from build123d import *

# Parameters (mm, degrees)
BOSS_EXTRUDE1_DEPTH      = 10
BOSS_EXTRUDE1_DEPTH_BACK = 12
SKETCH1_W                = 70
SKETCH1_H                = 20
SKETCH1_R                = 2.187999439
SKETCH1_R_2              = 2.181063018
HOLE1_D                  = 6
HOLE1_CBORE_D            = 9.5
HOLE1_CBORE_DEPTH        = 8.5
CHAMFER1_SIZE            = 2


with BuildPart() as part:
    # Sketch1 → Boss-Extrude1 (new, two sides: drawn at the far end of the back side and taken through both)
    with BuildSketch(Plane.XY.offset(-BOSS_EXTRUDE1_DEPTH_BACK)):
        with Locations((2.309691162, 2.003205128)):
            Rectangle(SKETCH1_W, SKETCH1_H)
        with Locations((-24.690308838, 2.003205128)):
            Circle(SKETCH1_R, mode=Mode.SUBTRACT)
        with Locations((29.309691162, 2.003205128)):
            Circle(SKETCH1_R_2, mode=Mode.SUBTRACT)
    extrude(amount=BOSS_EXTRUDE1_DEPTH + BOSS_EXTRUDE1_DEPTH_BACK)

    # Hole1 (through all)
    with Locations(Plane.XY.offset(10)):
        with Locations((-24.690308838, 2.003205128), (29.309691162, 2.003205128)):
            CounterBoreHole(HOLE1_D / 2, HOLE1_CBORE_D / 2, HOLE1_CBORE_DEPTH)

    # Chamfer1
    chamfer1_edges = [part.edges().sort_by_distance(p)[0] for p in [
        (-32.690308838, 12.003205128, -1),
        (37.309691162, 12.003205128, -1),
        (37.309691162, -7.996794872, -1),
        (-32.690308838, -7.996794872, -1),
    ]]
    chamfer(chamfer1_edges, length=CHAMFER1_SIZE)


solid = part.part
Design review of the part built by this model. Coordinates are the model's own, in mm. A direction names the side the tool comes from. Coordinates: 2 decimals unless noted, no trailing zeros. Order: outer loops, then holes, each group sorted by start corner. A loop starts at its lowest first (then second) coordinate and runs counter-clockwise, first axis right, second up.
Item 1: Take a section at A-A, the plane y = 3.25. Write out the cut boundary in (x, z).
Item 2: For pin 1 Ø8 at (x, y) = (-24.69, 2) entering from +Z; pin 2 Ø5 at (x, y) = (-23, 0) entering from +Z, all flat-tipped, find the tip position at first contact; note any pin that passes through.
Item 3: The part is to be moulded in two halves that separate along Y. For faces 3 (the flat face through (-23.7, -1.1, 1.5)), 4 (the flat face through (-31.676, 11.017, -1.154)), 5 (the flat face through (-31.676, -7.011, -1.154)), say which applies: pulls with the +Y half, pulls with the -Y half, needs draft (parallel to the pull), parting line crosses it, or undercut.
Item 4: Take a section at C-C, the plane z = 3.5. Write out the cut boundary in (x, y).
Item 5: For line 1 (X direction, y = 1.25, z = 0); line 2 (X direction, y = 3, z = 9.25); line 3 (Z direction, x = 25, y = 3.25), list the stretches that pass through material, from the lowest coordinate up.
Item 6: For faces 1 (the cylindrical face through (26.54, 0.85, -5.34)), 2 (the cylindrical face through (25.54, -0.89, 5.81)), list the 3-axis set-ups (+Z, -Z, +X, -X, +Y, -Y) from which the entire face can be reached by the end or side of a thin tool; tool diameter is ignored.
Item 7: Take a section at B-B, the plane z = -3.75. Write out the cut boundary in (x, y).
The answers:
1. outline: (-32.69, -12) - (-27.42, -12) - (-27.42, 1.5) - (-29.27, 1.5) - (-29.27, 10) - (-32.69, 10) - close; (-21.96, -12) - (26.58, -12) - (26.58, 1.5) - (24.73, 1.5) - (24.73, 10) - (-20.11, 10) - (-20.11, 1.5) - (-21.96, 1.5) - close; (32.04, -12) - (37.31, -12) - (37.31, 10) - (33.89, 10) - (33.89, 1.5) - (32.04, 1.5) - close
2. pin 1: stops at z = 1.5
2. pin 2: stops at z = 10
3. face 3: undercut
3. face 4: pulls with the +Y half
3. face 5: pulls with the -Y half
4. outline: (-32.69, -6) - (-30.69, -8) - (35.31, -8) - (37.31, -6) - (37.31, 10) - (35.31, 12) - (-30.69, 12) - (-32.69, 10) - close; hole circle Ø9.5 at (-24.69, 2); hole circle Ø9.5 at (29.31, 2)
5. line 1: x = -32.69 to -27.59, -21.79 to 26.41, 32.21 to 37.31
5. line 2: x = -32.69 to -29.33, -20.05 to 24.67, 33.95 to 37.31
5. line 3: z = -12 to 1.5
6. face 1: +Z, -Z
6. face 2: +Z
7. outline: (-32.69, -6) - (-30.69, -8) - (35.31, -8) - (37.31, -6) - (37.31, 10) - (35.31, 12) - (-30.69, 12) - (-32.69, 10) - close; hole circle Ø6 at (-24.69, 2); hole circle Ø6 at (29.31, 2)
